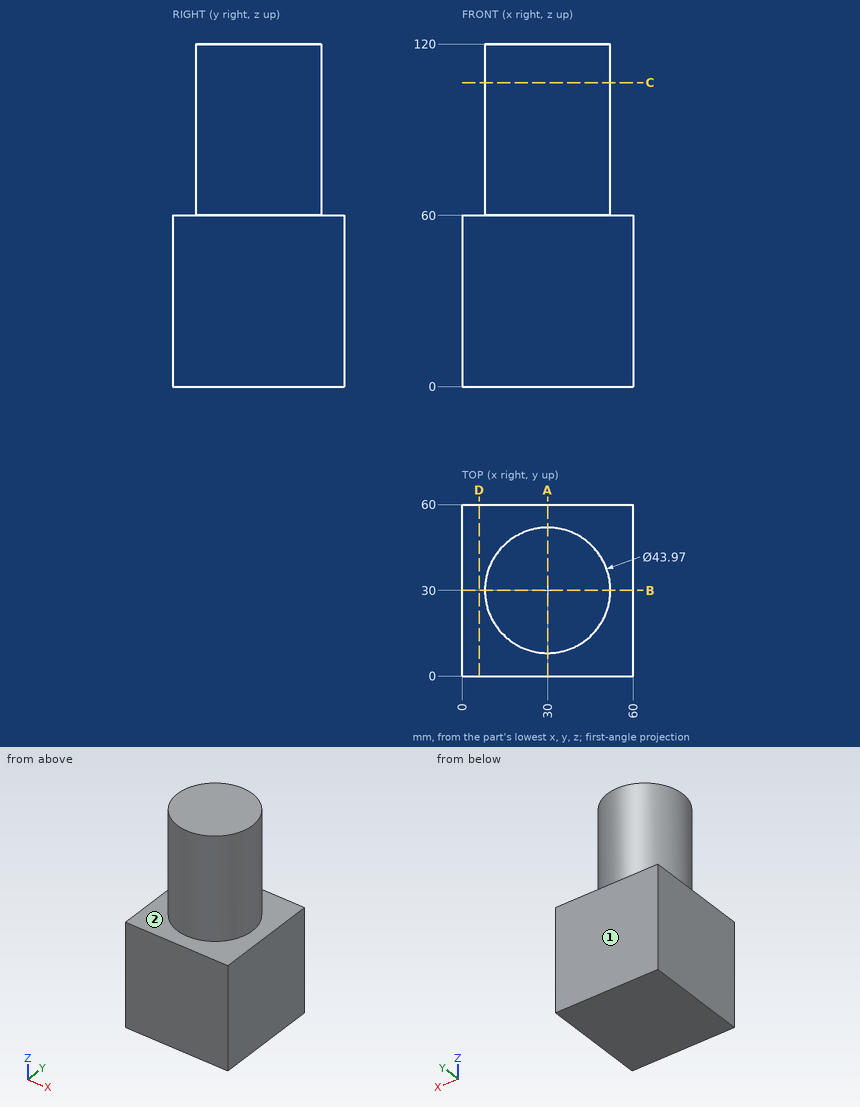
The figure shows three views and two pictorial views of one solid part (mm, origin at its lowest corner). Answer the questions. A direction names the side the tool comes from. Coordinates: 2 decimals unless noted, no trailing zeros. Loops run counter-clockwise (first coordinate to the right, second up) from the corner with the lowest first, then second, coordinate; pieces in that order, holes last. Notation, with made-up numbers: (83, -18) -> (88, -18) arc R11 cw to (88, -1) -> close; hole circle Ø5 at (-29, 0). An arc over 180 degrees is marked (long way). Write item = value, one per line. Start each with the question number.
1) A cutting plane is placed at C-C (z = 106.5). Give the vertices of the cut face in (x, y) (1 decimal), then the cut area to 3 significant figures.
2) Straight lines are drawn through the part: line 1 (Z direction, x = 15, y = 50.5); line 2 (X direction, y = 27, z = 104); line 3 (X direction, y = 19.5, z = 72.5) (1 decimal). For each, find the intervals that lie inside material, in ascending order. Write a range as from..to.
3) A tool of negligible diameter and unlimited length cuts with its end or side. For the marked faces 1 and 2, from which of +Z, -Z, +X, -X, +Y, -Y can it reach the whole face along a straight path? Write none if from no direction.
4) Given pin 1 Ø10 at (y, z) = (30.5, 69.5) entering from +X (1 decimal); pin 2 Ø3 at (y, z) = (37.5, 76.5) entering from +X; pin 3 Ø3 at (y, z) = (30.5, 64.5) entering from -X (1 decimal), each flat-ended and moving along its own axis, determine where each tip first touches the part or whether it passes through.
5) A cutting plane is placed at A-A (x = 30). Give the vertices of the cut face in (y, z) (1 decimal).
6) A cutting plane is placed at D-D (x = 6). Give the vertices of the cut face in (y, z).
Responses:
q1.outline = circle Ø44 at (30, 30)
q1.area = 1,520 mm²
q2.line_1 = 0..60
q2.line_2 = 8.22..51.78
q2.line_3 = 10.7..49.3
q3.face_1 = +Z, -Z, +X, -X, +Y
q3.face_2 = +Z
q4.pin_1 = 52
q4.pin_2 = 51.15
q4.pin_3 = 8
q5.outline = (0, 0) -> (60, 0) -> (60, 60) -> (52, 60) -> (52, 120) -> (8, 120) -> (8, 60) -> (0, 60) -> close
q6.outline = (0, 0) -> (60, 0) -> (60, 60) -> (0, 60) -> close
